from build123d import *

# Parameters (mm, degrees)
SKETCH1_R           = 8
BASEHEAD_DEPTH      = 10
SKETCH2_R           = 5
BASEBODY_DEPTH      = 50
HEXAGONSOCKET_DEPTH = 5
TOPFILLET_R         = 1.25
CHAMFER1_SIZE       = 0.4


with BuildPart() as part:
    # Sketch1 → BaseHead (new body)
    with BuildSketch(Plane(origin=(0, 0, 0), x_dir=(0, 0, -1), z_dir=(1, 0, 0))):
        Circle(SKETCH1_R)
    extrude(amount=BASEHEAD_DEPTH)

    # Sketch2 → BaseBody (add)
    with BuildSketch(Plane(origin=(10, 0, 0), x_dir=(0, 0, -1), z_dir=(1, 0, 0))):
        Circle(SKETCH2_R)
    extrude(amount=BASEBODY_DEPTH)

    # Sketch3 → HexagonSocket (cut)
    with BuildSketch(Plane(origin=(0, 0, 0), x_dir=(0, 0, -1), z_dir=(1, 0, 0))):
        Polygon((4.618802154, 0), (2.309401077, 4), (-2.309401077, 4), (-4.618802154, 0), (-2.309401077, -4), (2.309401077, -4), align=None)
    extrude(amount=HEXAGONSOCKET_DEPTH, mode=Mode.SUBTRACT)

    # Sketch4 → Cut-Revolve1 (revolve, cut)
    with BuildSketch(Plane(origin=(-4.19613823, 0.75, 0), x_dir=(-1, 0, 0), z_dir=(0, 0, 1)), mode=Mode.PRIVATE) as cut_revolve1_sk:
        Polygon((-9.19613823, 4.75), (-11.505539306, 0.75), (-9.19613823, 0.75), align=None)
    revolve(cut_revolve1_sk.sketch.rotate(Axis((0.838992387, 0, 0), (-1, 0, 0)), 90), axis=Axis((0.838992387, 0, 0), (-1, 0, 0)), mode=Mode.SUBTRACT)

    # TopFillet
    topfillet_edges = [part.edges().sort_by_distance(p)[0] for p in [
        (0, 0, 8),
    ]]
    fillet(topfillet_edges, radius=TOPFILLET_R)

    # Chamfer1
    chamfer1_edges = [part.edges().sort_by_distance(p)[0] for p in [
        (60, 0, 5),
    ]]
    chamfer(chamfer1_edges, length=CHAMFER1_SIZE)


solid = part.part
For this review, take the finished solid that the model builds, in its own axes (mm). A direction names the side the tool comes from. Round coordinates to 2 decimals unless told otherwise and drop trailing zeros. Order: outer loops, then holes, each group sorted by start corner. A loop starts at its lowest first (then second) coordinate and runs counter-clockwise, first axis right, second up. Notation, with made-up numbers: M 34.5,-38.5 L 65.5,-38.5 A27 ccw 65.5,-4.5 Z; hole C 45.5,12 d10. An arc over 180 degrees is marked long. Use a Markdown table: item, result. Add a question column.
Item 1: Add section A-A, the plane x = 42.5. Give the boundary of the cut face in (y, z), then the cut area to 3 significant figures.
Item 2: To check wall thickness, follow line 1 along X through (y, z) = (-5, 1.5); line 2 along Y through (x, z) = (40, 0.25); line 3 along Z through (x, y) = (3, 4.5). State the ranges of each line that lie inside material, in increasing order.
Item 3: Tool access review of faces 1 (the flat face through (5, -3.6, 2.1)), 2 (the cylindrical face through (5.56, -7.81, 1.73)), 3 (the flat face through (10, 0.1, -5.2)): name each direction out of +Z, -Z, +X, -X, +Y, -Y from which nothing blocks a thin tool from reaching the whole face with its end or side.
Item 4: Insertion check: pin 1 (2 mm diameter, centred on y = -2.5, z = -1, fed in from -X); pin 2 (1 mm diameter, centred on x = 47, z = -6, fed in from +Y); pin 3 (3 mm diameter, centred on x = 8.5, z = -4, fed in from -Y); pin 4 (1 mm diameter, centred on x = 6.5, z = 3, fed in from +Y). Each pin has a flat end and moves straight along its axis. Give the tip position at first contact, or say it passes through.
Item 5: Mouldability with a two-part tool opening along Z and no side actions: class faces 4 (the flat face through (0, -4.4, 0.1)), 5 (the cylindrical face through (34.45, -4.88, 1.08)), 6 (the flat face through (2.46, 1.97, -3.48)) as released by +Z, released by -Z, zero draft, split by the parting line, or undercut.
Geometry results:
| question | item | result |
|---|---|---|
| 1 | outline | C 0,0 d10 |
| 1 | area | 78.5 mm² |
| 2 | line 1 | x = 0 to 10 |
| 2 | line 2 | y = -4.99 to 4.99 |
| 2 | line 3 | z = -6.61 to 6.61 |
| 3 | face 1 | -X |
| 3 | face 2 | +X, -X |
| 3 | face 3 | +X |
| 4 | pin 1 | stops at x = 5.18 |
| 4 | pin 2 | passes through |
| 4 | pin 3 | stops at y = -7.6 |
| 4 | pin 4 | stops at y = 7.6 |
| 5 | face 4 | zero draft |
| 5 | face 5 | split by the parting line |
| 5 | face 6 | undercut |
